Part model, mm, in its own coordinate system. Round coordinates to 2 decimals unless told otherwise and drop trailing zeros. Loops run counter-clockwise (first coordinate to the right, second up) from the corner with the lowest first, then second, coordinate; pieces in that order, holes last. Notation, with made-up numbers: M 35.25,18 L 71.25,18 A25 ccw 71.25,44 Z; hole C 47,45.25 d11. An arc over 180 degrees is marked long. Answer as CSV lines item,"result". Start each with the question number.
Item 1: Band-saw the part on A-A (x = 0). Give the cut face in (y, z) (3 decimals), and give its area (3 significant figures).
Item 2: Band-saw the part on D-D (x = 13). Give the cut face in (y, z) (3 decimals), and give its area (3 significant figures).
Item 3: Mould opens along X. For faces 1 (the cylindrical face through (-6.085, -0.07, -32.441)), 2 (the cylindrical face through (0.4, 0.1, -44.5)), 3 (the flat face through (0, 0, 24.505)) say: pulls with the +X half, pulls with the -X half, needs draft (parallel to the pull), parting line crosses it, or undercut.
Item 4: Wall check: line 1 (Z direction, x = 6, y = 0) (3 decimals); line 2 (Z direction, x = 1, y = 4) (3 decimals); line 3 (X direction, y = 2.5, z = -21.5). Give the ranges that are in metal, low to high.
Item 5: Drop flat-ended pins along their axis: pin 1 Ø2 at (x, y) = (13, 3) entering from -Z (3 decimals); pin 2 Ø4 at (x, y) = (-1.5, -3) entering from -Z (3 decimals). Give the stop position or say it passes through.
Item 6: Band-saw the part on B-B (y = -0.25). Give the cut face in (x, z) (3 decimals), and give its area (3 significant figures).
Item 7: Band-saw the part on C-C (z = -20). Give the cut face in (x, y).
```python
from build123d import *

# Parameters (mm, degrees)
SKETCH_1_R      = 10
EXTRUDE_1_DEPTH = 5


with BuildPart() as part:
    # 草图1 → 凸台-拉伸1 (new, symmetric)
    with BuildSketch(Plane(origin=(0, 0, 0), x_dir=(1, 0, 0), z_dir=(0, 1, 0))):
        with BuildLine():
            Line((-20, -24.505), (20, -24.505))
            Line((20, -24.505), (20, 24.505))
            ThreePointArc((20, 24.505), (0, 44.505), (-20, 24.505))
            Line((-20, 24.505), (-20, -24.505))
        make_face()
        with Locations(Location((0, 24.505, 0), (0, 0, 270))):
            Circle(SKETCH_1_R, mode=Mode.SUBTRACT)
    extrude(amount=EXTRUDE_1_DEPTH, both=True)


solid = part.part
```
Answer block:
1,outline,"M -5,-44.505 L 5,-44.505 L 5,-34.505 L -5,-34.505 Z; M -5,-14.505 L 5,-14.505 L 5,24.505 L -5,24.505 Z"
1,area,"490 mm^2"
2,outline,"M -5,-39.704 L 5,-39.704 L 5,24.505 L -5,24.505 Z"
2,area,"642 mm^2"
3,face 1,"undercut"
3,face 2,"parting line crosses it"
3,face 3,"needs draft"
4,line 1,"z = -43.584 to -32.505, -16.505 to 24.505"
4,line 2,"z = -44.48 to -34.455, -14.555 to 24.505"
4,line 3,"x = -20 to -9.54, 9.54 to 20"
5,pin 1,"stops at z = -40.505"
5,pin 2,"stops at z = -44.505"
6,outline,"M -20,-24.505 A20 ccw 20,-24.505 L 20,24.505 L -20,24.505 Z; hole C 0,-24.505 d20"
6,area,"2,270 mm^2"
7,outline,"M -20,-5 L -8.93,-5 L -8.93,5 L -20,5 Z; M 8.93,-5 L 20,-5 L 20,5 L 8.93,5 Z"
